The drawing under review shows one solid part. Ordinate dimensions are in mm from its lowest x, y, z. A direction names the side the tool comes from. Round coordinates to 2 decimals unless told otherwise and drop trailing zeros. Write each loop counter-clockwise with the first axis right and the second up, starting at its lowest first coordinate (ties: lowest second). Pieces come first, ordered by that corner, then holes. Notation, with made-up numbers: M 21.5,87 L 28.5,87 A31 ccw 28.5,125 Z; hole C 9,37 d8. An arc over 180 degrees is marked long. One line per item, written item: value. Start each with the question number.
1) Take a section at D-D, the plane y = 5.5. Write out the cut boundary in (x, z), and give its area (3 significant figures).
2) Mouldability with a two-part tool opening along X and no side actions: class the marked faces 3, 4 and 5 as +X half, -X half, draft (parallel to the pull), parting line (faces both ways), or undercut.
3) Take a section at C-C, the plane z = 29. Write out the cut boundary in (x, y).
4) Wall thickness on probe 1 along X at (y, z) = (15, 15.4); probe 2 along X at (y, z) = (9.5, 31.5); probe 3 along X at (y, z) = (15.5, 16): over which ranges is each line inside the solid? List them lowest first.
5) Take a section at B-B, the plane x = 30. Write out the cut boundary in (y, z).
6) Tool access review of the marked faces 1 and 2: name each direction out of +Z, -Z, +X, -X, +Y, -Y from which nothing blocks a thin tool from reaching the whole face with its end or side.
7) Take a section at A-A, the plane y = 17.5. Write out the cut boundary in (x, z), and give its area (3 significant figures).
8) For P1, Ø10, axis at x = 22.5, y = 17.5, coming from the -Z side; P2, Ø1.1, axis at x = 30, z = 15.5, coming from the +Y side; P3, Ø12, axis at x = 16.5, z = 29, coming from the -Y side, all flat-tipped, find the tip position at first contact; note any pin that passes through.
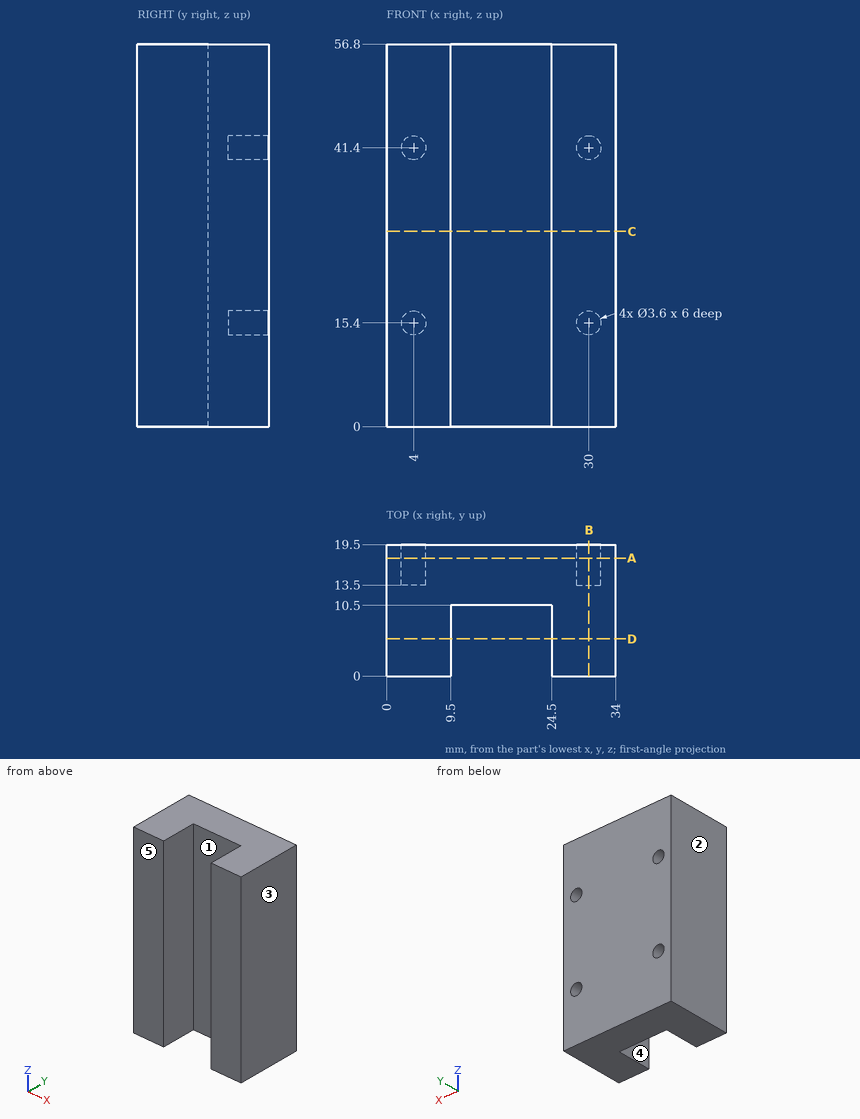
Checked values:
1. outline: M 0,0 L 9.5,0 L 9.5,56.8 L 0,56.8 Z; M 24.5,0 L 34,0 L 34,56.8 L 24.5,56.8 Z
1. area: 1,080 mm2
2. face 3: +X half
2. face 4: undercut
2. face 5: draft
3. outline: M 0,0 L 9.5,0 L 9.5,10.5 L 24.5,10.5 L 24.5,0 L 34,0 L 34,19.5 L 0,19.5 Z
4. probe 1: x = 0 to 2.2, 5.8 to 28.2, 31.8 to 34
4. probe 2: x = 0 to 9.5, 24.5 to 34
4. probe 3: x = 0 to 2.3, 5.7 to 28.3, 31.7 to 34
5. outline: M 0,0 L 19.5,0 L 19.5,13.6 L 13.5,13.6 L 13.5,17.2 L 19.5,17.2 L 19.5,39.6 L 13.5,39.6 L 13.5,43.2 L 19.5,43.2 L 19.5,56.8 L 0,56.8 Z
6. face 1: +Z, -Z, -Y
6. face 2: +Z, -Z, -X, +Y, -Y
7. outline: M 0,0 L 34,0 L 34,56.8 L 0,56.8 Z; hole C 4,15.4 d3.6; hole C 4,41.4 d3.6; hole C 30,15.4 d3.6; hole C 30,41.4 d3.6
7. area: 1,890 mm2
8. P1: stops at z = 0
8. P2: stops at y = 13.5
8. P3: stops at y = 10.5
